Check sheet for the drawn part. Datum: minimum x, y, z corner. Units: mm. A direction names the side the tool comes from. Round coordinates to 2 decimals unless told otherwise and drop trailing zeros. Write each loop counter-clockwise with the first axis right and the second up, starting at its lowest first coordinate (ties: lowest second). Pieces come first, ordered by that corner, then holes.
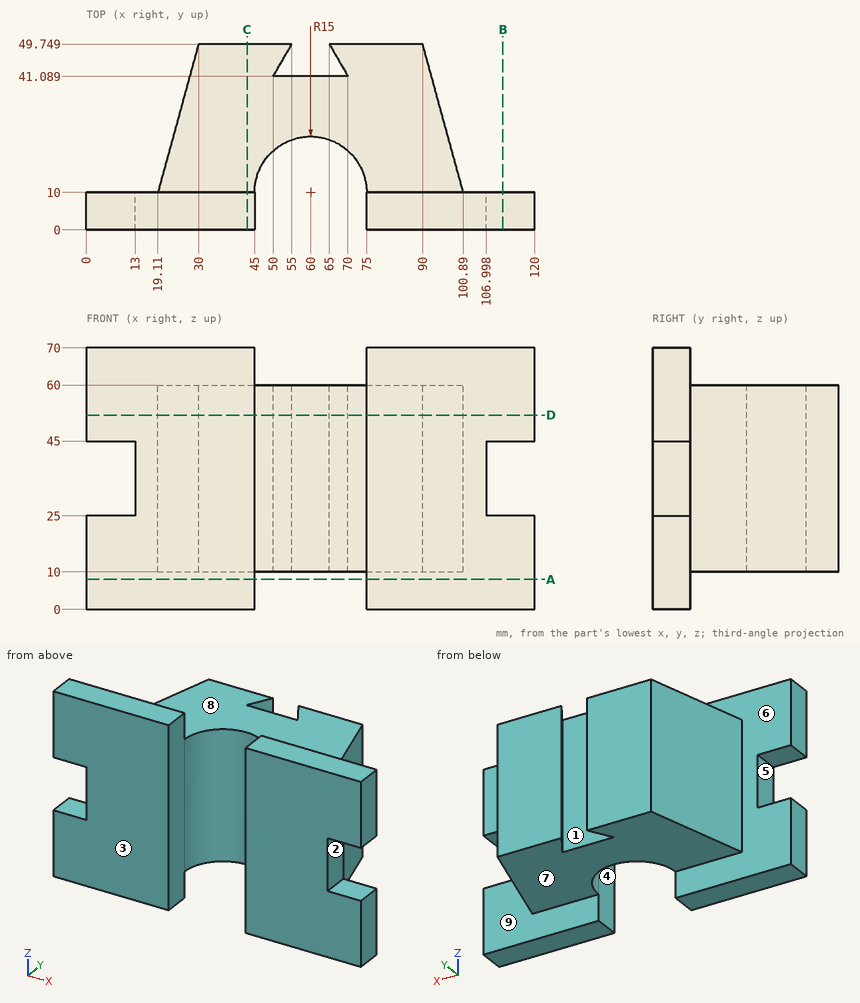
1. Release check for a two-part mould opening along X. For the marked faces 1, 2, 3 and 4 record: released by +X, released by -X, zero draft, split by the parting line, or undercut.
2. Sectioned sample at C-C, the plane x = 43. Enter the section's corners in (y, z), plus the area to 3 significant figures.
3. Sectioned sample at B-B, the plane x = 111.5. Enter the section's corners in (y, z), plus the area to 3 significant figures.
4. Go/stop test with flat-tipped pins: pin 1 (3 mm diameter, centred on x = 96.5, y = 28, fed in from +Z); pin 2 (5 mm diameter, centred on x = 99, y = 19, fed in from -Z); pin 3 (5 mm diameter, centred on y = 5.5, z = 28, fed in from +X); pin 4 (8 mm diameter, centred on x = 114, y = 3, fed in from -Z). Record where each tip stops, or that it passes through.
5. Scan lines: line 1 along X through (y, z) = (3, 54); line 2 along Y through (x, z) = (9, 8); line 3 along Z through (x, y) = (54, 36.5). Record each from-to range of solid material in increasing order.
6. Sectioned sample at A-A, the plane z = 8. Enter the section's corners in (x, y).
7. Set-up check for the marked faces 5, 6, 7, 8 and 9: record each of +Z, -Z, +X, -X, +Y, -Y from which the full face is reachable in a straight line by a thin tool's end or side.
8. Sectioned sample at D-D, the plane z = 52. Enter the section's corners in (x, y).
Computed values:
1. face 1: undercut
1. face 2: released by +X
1. face 3: zero draft
1. face 4: undercut
2. outline: (0, 0) - (10, 0) - (10, 10) - (49.75, 10) - (49.75, 60) - (10, 60) - (10, 70) - (0, 70) - close
2. area: 2,690 mm2
3. outline: (0, 0) - (10, 0) - (10, 25) - (0, 25) - close; (0, 45) - (10, 45) - (10, 70) - (0, 70) - close
3. area: 500 mm2
4. pin 1: stops at z = 60
4. pin 2: stops at z = 10
4. pin 3: stops at x = 107
4. pin 4: stops at z = 0
5. line 1: x = 0 to 45, 75 to 120
5. line 2: y = 0 to 10
5. line 3: z = 10 to 60
6. outline: (0, 0) - (45, 0) - (45, 10) - (0, 10) - close; (75, 0) - (120, 0) - (120, 10) - (75, 10) - close
7. face 5: -X, +Y, -Y
7. face 6: -X, +Y
7. face 7: -Z, +X, -X, +Y
7. face 8: +Z, +X, -X, +Y
7. face 9: +X, +Y
8. outline: (0, 0) - (45, 0) - (45, 10) arc R15 cw to (75, 10) - (75, 0) - (120, 0) - (120, 10) - (100.89, 10) - (90, 49.75) - (65, 49.75) - (70, 41.09) - (50, 41.09) - (55, 49.75) - (30, 49.75) - (19.11, 10) - (0, 10) - close
